Work out the finished part from the listing and answer in its coordinate system (mm). A direction names the side the tool comes from. Round coordinates to 2 decimals unless told otherwise and drop trailing zeros. Order: outer loops, then holes, each group sorted by start corner. A loop starts at its lowest first (then second) coordinate and runs counter-clockwise, first axis right, second up. Notation, with made-up numbers: (65.5, 80.5) -> (110.5, 80.5) arc R12 cw to (110.5, 101.5) -> close; hole circle Ø1 at (3, 36.5). An arc over 180 degrees is marked (long way). Use one line per item in the form item = value.
```python
from build123d import *

# Parameters (mm, degrees)
BASE_PLATE_PROFILE_SKETCH_R = 12.5
BASE_LUG_PLATE_DEPTH        = 30
HOLE_BOSS_SKETCH_R          = 15
HOLE_BOSS_PADS_DEPTH        = 6
MOUNTING_HOLES_SKETCH_R     = 12.5
MOUNTING_HOLES_DEPTH        = 150.506388346
FLANGE_PAD_SKETCH_W         = 57.5
FLANGE_PAD_SKETCH_H         = 120
FLANGE_PAD_DEPTH            = 6
CONNECTING_ARM_SKETCH_W     = 30
CONNECTING_ARM_SKETCH_H     = 120
CONNECTING_ARM_DEPTH        = 166
VERTICAL_WEB_SKETCH_R       = 57.5
VERTICAL_WEB_SKETCH_R_2     = 37.5
VERTICAL_WEB_DEPTH          = 60
ARM_TRIM_CUT_DEPTH          = 317.920195248
HUB_NECK_DEPTH              = 13
HUB_CYLINDER_SKETCH_R       = 37.5
HUB_CYLINDER_SKETCH_R_2     = 22.5
HUB_CYLINDER_DEPTH          = 25
HUB_BORE_SKETCH_R           = 22.5
HUB_BORE_DEPTH              = 318.107730117


with BuildPart() as part:
    # Base Plate Profile Sketch → Base Lug Plate (new body)
    with BuildSketch(Plane.XY):
        with BuildLine():
            Line((108.8125, 60), (108.8125, -60))
            ThreePointArc((108.8125, -60), (72.8125, -96), (36.8125, -60))
            Line((36.8125, -60), (-66.25, -60))
            Line((-66.25, -60), (-66.25, 60))
            Line((-66.25, 60), (36.8125, 60))
            ThreePointArc((36.8125, 60), (72.8125, 96), (108.8125, 60))
        make_face()
        with Locations((72.8125, 60)):
            Circle(BASE_PLATE_PROFILE_SKETCH_R, mode=Mode.SUBTRACT)
        with Locations((72.8125, -60)):
            Circle(BASE_PLATE_PROFILE_SKETCH_R, mode=Mode.SUBTRACT)
    extrude(amount=BASE_LUG_PLATE_DEPTH)

    # Hole Boss Sketch → Hole Boss Pads (add)
    with BuildSketch(Plane.XY.offset(30)):
        with Locations((72.8125, 60)):
            Circle(HOLE_BOSS_SKETCH_R)
        with Locations((72.8125, -60)):
            Circle(HOLE_BOSS_SKETCH_R)
    extrude(amount=HOLE_BOSS_PADS_DEPTH)

    # Mounting Holes Sketch → Mounting Holes (cut, through all)
    with BuildSketch(Plane(origin=(0, 0, 0), x_dir=(-1, 0, 0), z_dir=(0, 0, -1))):
        with Locations((-72.8125, 60)):
            Circle(MOUNTING_HOLES_SKETCH_R)
        with Locations((-72.8125, -60)):
            Circle(MOUNTING_HOLES_SKETCH_R)
    extrude(amount=-MOUNTING_HOLES_DEPTH, mode=Mode.SUBTRACT)

    # Flange Pad Sketch → Flange Pad (add)
    with BuildSketch(Plane(origin=(0, 0, 0), x_dir=(-1, 0, 0), z_dir=(0, 0, -1))):
        with Locations((37.5, 0)):
            Rectangle(FLANGE_PAD_SKETCH_W, FLANGE_PAD_SKETCH_H)
    extrude(amount=FLANGE_PAD_DEPTH)

    # Connecting Arm Sketch → Connecting Arm (add)
    with BuildSketch(Plane.XY.offset(30)):
        with Locations((-51.25, 0)):
            Rectangle(CONNECTING_ARM_SKETCH_W, CONNECTING_ARM_SKETCH_H)
    extrude(amount=CONNECTING_ARM_DEPTH)

    # Vertical Web Sketch → Vertical Web (add, symmetric)
    with BuildSketch(Plane(origin=(0, 0, 0), x_dir=(1, 0, 0), z_dir=(0, 1, 0))):
        with Locations((-8.75, -196)):
            Circle(VERTICAL_WEB_SKETCH_R)
        with Locations((-8.75, -196)):
            Circle(VERTICAL_WEB_SKETCH_R_2, mode=Mode.SUBTRACT)
    extrude(amount=VERTICAL_WEB_DEPTH, both=True)

    # Arm Trim Sketch → Arm Trim Cut (cut, through all)
    with BuildSketch(Plane(origin=(0, 60, 0), x_dir=(1, 0, 0), z_dir=(0, 1, 0))):
        with BuildLine():
            Line((-36.25, -196), (-36.25, -170.504902432))
            ThreePointArc((-36.25, -170.504902432), (-43.660600109, -182.306936062), (-46.25, -196))
            Line((-46.25, -196), (-36.25, -196))
        make_face()
    extrude(amount=-ARM_TRIM_CUT_DEPTH, mode=Mode.SUBTRACT)

    # Hub Neck Sketch → Hub Neck (add, symmetric)
    with BuildSketch(Plane(origin=(0, 0, 0), x_dir=(1, 0, 0), z_dir=(0, 1, 0))):
        with BuildLine():
            Line((-141.503483954, -89.145484499), (-66.25, -196))
            Line((-66.25, -196), (-66.25, 6))
            Line((-66.25, 6), (-136.449661852, -44.296082333))
            ThreePointArc((-136.449661852, -44.296082333), (-148.385562866, -62.269844624), (-145.38363754, -83.635946473))
            Line((-145.38363754, -83.635946473), (-141.503483954, -89.145484499))
        make_face()
    extrude(amount=HUB_NECK_DEPTH, both=True)

    # Hub Cylinder Sketch → Hub Cylinder (add, symmetric)
    with BuildSketch(Plane(origin=(0, 0, 0), x_dir=(1, 0, 0), z_dir=(0, 1, 0))):
        with Locations(Location((-118.75, -69, 0), (0, 0, 270))):
            Circle(HUB_CYLINDER_SKETCH_R)
        with Locations(Location((-118.75, -69, 0), (0, 0, 270))):
            Circle(HUB_CYLINDER_SKETCH_R_2, mode=Mode.SUBTRACT)
    extrude(amount=HUB_CYLINDER_DEPTH, both=True)

    # Hub Bore Sketch → Hub Bore (cut, through all)
    with BuildSketch(Plane(origin=(0, 13, 0), x_dir=(1, 0, 0), z_dir=(0, 1, 0))):
        with Locations(Location((-118.75, -69, 0), (0, 0, 270))):
            Circle(HUB_BORE_SKETCH_R)
    extrude(amount=-HUB_BORE_DEPTH, mode=Mode.SUBTRACT)


solid = part.part
```
Item 1: Flat-ended cylindrical pins translate along their axes: P1, Ø19.5, axis at x = -98.5, z = 64.5, coming from the +Y side; P2, Ø5, axis at x = -85.5, y = -15, coming from the +Z side; P3, Ø19.5, axis at x = -113, z = 84, coming from the -Y side; P4, Ø22.5, axis at x = 72.81, y = 60, coming from the -Z side. Find the tip coordinate at first contact, or state that the pin passes through.
Findings:
P1 = 25
P2 = 170.8
P3 = -25
P4 = through
Item 2: The part is cut by section A-A, the plane y = -21. Give the vertices of the cut face in (x, z).
Findings:
outline = circle Ø75 at (-118.75, 69); (-66.25, -6) -> (-8.75, -6) -> (-8.75, 0) -> (108.81, 0) -> (108.81, 30) -> (-36.25, 30) -> (-36.25, 145.5) arc R57.5 ccw (long way) to (-66.25, 196) -> close; hole circle Ø45 at (-118.75, 69); hole circle Ø75 at (-8.75, 196)
Item 3: Determine the mould class of faces 1 (the flat face through (-66.25, -37, 94)), 2 (the flat face through (-85, 13, 94)), 3 (the cylindrical face through (69.561, -74.643, 32.958)), 4 (the cylindrical face through (69.561, 45.357, 32.958)) for opening direction Y: released by +Y, released by -Y, zero draft, split by the parting line, or undercut.
Findings:
face_1 = zero draft
face_2 = released by +Y
face_3 = undercut
face_4 = undercut
Item 4: The part is cut by section C-C, the plane x = 21. Give the vertices of the cut face in (y, z), and give its area (3 significant figures).
Findings:
outline = (-60, 0) -> (60, 0) -> (60, 30) -> (-60, 30) -> close; (-60, 146.79) -> (60, 146.79) -> (60, 173.17) -> (-60, 173.17) -> close; (-60, 218.83) -> (60, 218.83) -> (60, 245.21) -> (-60, 245.21) -> close
area = 9,930 mm^2
Item 5: The part is cut by section D-D, the plane z = 212.5. Give the vertices of the cut face in (x, y).
Findings:
outline = (-63.83, -60) -> (-42.42, -60) -> (-42.42, 60) -> (-63.83, 60) -> close; (24.92, -60) -> (46.33, -60) -> (46.33, 60) -> (24.92, 60) -> close
Item 6: The part is cut by section B-B, the plane y = 0. Give the vertices of the cut face in (x, z), and give its area (3 significant figures).
Findings:
outline = (-130.65, 104.56) arc R37.5 ccw to (-118.59, 31.5) -> (-66.25, -6) -> (-8.75, -6) -> (-8.75, 0) -> (108.81, 0) -> (108.81, 30) -> (-36.25, 30) -> (-36.25, 145.5) arc R57.5 ccw (long way) to (-66.25, 196) -> close; hole circle Ø45 at (-118.75, 69); hole circle Ø75 at (-8.75, 196)
area = 23,800 mm^2
Item 7: For faces 5 (the flat face through (-135, 25, 85)), 6 (the flat face through (69.4, 72.3, 36)), 7 (the flat face through (51, 1, 0)), determine the directions among +Z, -Z, +X, -X, +Y, -Y from which every point of the face is accessible in a straight line to the end or side of a thin tool.
Findings:
face_5 = +Z, -Z, -X, +Y
face_6 = +Z, +X, +Y, -Y
face_7 = -Z, +X, +Y, -Y
Item 8: Consider line 1 along X through (y, z) = (20, 69); line 2 along Z through (x, y) = (-8, -23); line 3 along Z through (x, y) = (-21, 50.5). Determine where each line is inside the solid, lowest interval first.
Findings:
line_1 = -156.25 to -141.25, -96.25 to -81.25, -66.25 to -36.25
line_2 = 0 to 30, 138.5 to 158.51, 233.49 to 253.5
line_3 = -6 to 30, 139.82 to 160.56, 231.44 to 252.18
